Input: dimensioned drawing with shaded views. Units: mm. Origin: part minimum x, y, z. A direction names the side the tool comes from. Give positions to 0.01 mm unless a question says otherwise; leave off trailing zeros. Write each loop counter-clockwise with the first axis right and the second up, starting at its lowest first coordinate (ties: lowest second). Pieces come first, ordered by that corner, then holes. Notation, with made-up numbers: (19.25, 75) -> (37.25, 75) arc R19 cw to (37.25, 103) -> close; hole circle Ø9 at (45.25, 14). An arc over 180 degrees is marked (long way). Answer in a Markdown table with one row per item. Add a question column.
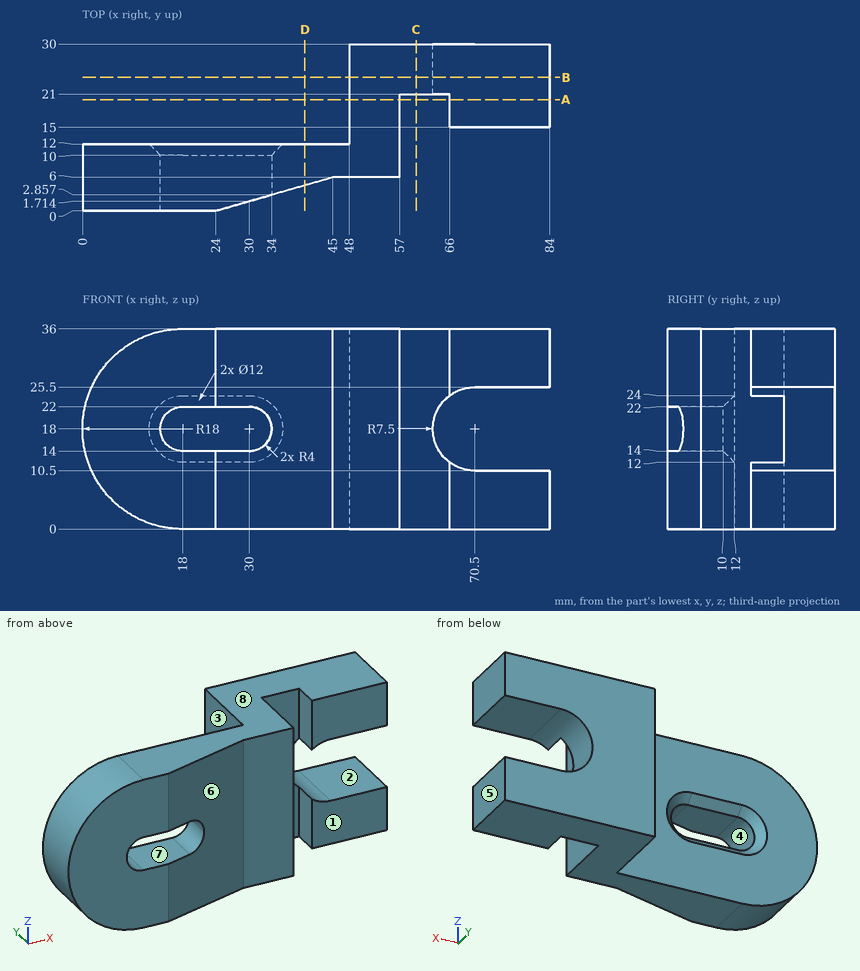
Q1. Pull-direction query (X, two-part tool) for the marked faces 6, 7 and 8; classes: +X half, -X half, draft (parallel to the pull), parting line (faces both ways), or undercut.
Q2. Contact query for flat-ended pins moving along their axis: pin 1 Ø6 at (x, z) = (52, 9) entering from -Y; pin 2 Ø8 at (y, z) = (4, 19) entering from -X; pin 3 Ø15 at (x, y) = (80.5, 21) entering from -Z; pin 4 Ø5.5 at (y, z) = (24.5, 24.5) entering from -X. Output: stop coordinate, or through.
Q3. Section A-A on y = 20. Return loops of the section in (x, z), and give its area (3 significant figures).
Q4. Line query: probe 1 along Z at (x, y) = (66, 21.75); probe 2 along X at (y, z) = (21.25, 12); probe 3 along Y at (x, z) = (19, 10). Output: solid intervals per line, ascending. Write a range as from..to.
Q5. Section B-B on y = 24. Return loops of the section in (x, z).
Q6. Section D-D on x = 40. Return loops of the section in (y, z).
Q7. Section C-C on x = 60. Return loops of the section in (y, z), and give its area (3 significant figures).
Q8. Access query for the marked faces 1, 2, 3, 4 and 5. Directions: +Z, -Z, +X, -X, +Y, -Y. A direction counts if a zero-diameter tool reaches every point of the face in a straight line with its end or side. Return the directions, or none.
Checks:
| question | item | result |
|---|---|---|
| 1 | face 6 | +X half |
| 1 | face 7 | undercut |
| 1 | face 8 | draft |
| 2 | pin 1 | y = 6 |
| 2 | pin 2 | x = 0 |
| 2 | pin 3 | z = 0 |
| 2 | pin 4 | x = 48 |
| 3 | outline | (48, 0) -> (57, 0) -> (57, 36) -> (48, 36) -> close; (66, 0) -> (84, 0) -> (84, 10.5) -> (70.5, 10.5) arc R7.5 cw to (66, 12) -> close; (66, 24) arc R7.5 cw to (70.5, 25.5) -> (84, 25.5) -> (84, 36) -> (66, 36) -> close |
| 3 | area | 706 mm^2 |
| 4 | probe 1 | 0..12, 24..36 |
| 4 | probe 2 | 48..66 |
| 4 | probe 3 | 0..12 |
| 5 | outline | (48, 0) -> (84, 0) -> (84, 10.5) -> (70.5, 10.5) arc R7.5 cw to (70.5, 25.5) -> (84, 25.5) -> (84, 36) -> (48, 36) -> close |
| 6 | outline | (4.57, 0) -> (12, 0) -> (12, 36) -> (4.57, 36) -> close |
| 7 | outline | (21, 0) -> (30, 0) -> (30, 36) -> (21, 36) -> close |
| 7 | area | 324 mm^2 |
| 8 | face 1 | +Z, -Z, +X, -Y |
| 8 | face 2 | +X, +Y, -Y |
| 8 | face 3 | +Z, -Z, -X, +Y |
| 8 | face 4 | +Y, -Y |
| 8 | face 5 | +Z, -Z, +X, +Y, -Y |
